Geometry: see drawing. Coordinates: mm, zero at the bounding-box minimum. A direction names the side the tool comes from. Round coordinates to 2 decimals unless told otherwise and drop trailing zeros. Order: outer loops, then holes, each group sorted by start corner. A loop starts at its lowest first (then second) coordinate and runs counter-clockwise, first axis right, second up.
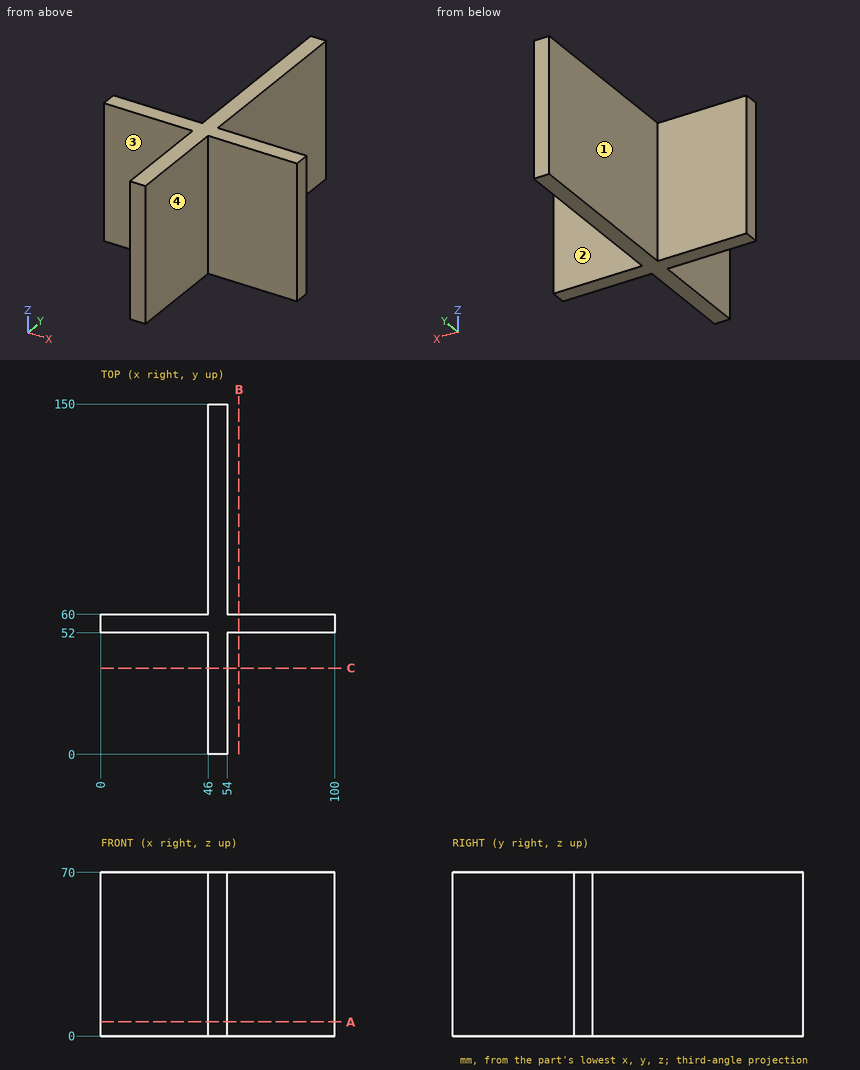
1. Section C-C on y = 37. Return loops of the section in (x, z).
2. Access query for the marked faces 1, 2, 3 and 4. Directions: +Z, -Z, +X, -X, +Y, -Y. A direction counts if a zero-diameter tool reaches every point of the face in a straight line with its end or side. Return the directions, or none.
3. Line query: line 1 along Y through (x, z) = (26.5, 63); line 2 along X through (y, z) = (96.5, 23). Output: solid intervals per line, ascending.
4. Section B-B on x = 59. Return loops of the section in (y, z).
5. Section A-A on z = 6. Return loops of the section in (x, y).
6. First-contact query: pin 1 (21 mm diameter, centred on y = 103, z = 44, fed in from -X); pin 2 (2 mm diameter, centred on x = 89, z = 43.5, fed in from +Y); pin 3 (3 mm diameter, centred on x = 85, z = 50, fed in from -Y). Flat tips, straight axial feed; report the tip coordinate or a pass-through.
Result:
1. outline: (46, 0) - (54, 0) - (54, 70) - (46, 70) - close
2. face 1: +Z, -Z, -X, +Y
2. face 2: +Z, -Z, +X, +Y
2. face 3: +Z, -Z, -X, -Y
2. face 4: +Z, -Z, +X, -Y
3. line 1: y = 52 to 60
3. line 2: x = 46 to 54
4. outline: (52, 0) - (60, 0) - (60, 70) - (52, 70) - close
5. outline: (0, 52) - (46, 52) - (46, 0) - (54, 0) - (54, 52) - (100, 52) - (100, 60) - (54, 60) - (54, 150) - (46, 150) - (46, 60) - (0, 60) - close
6. pin 1: stops at x = 46
6. pin 2: stops at y = 60
6. pin 3: stops at y = 52
